Geometry check sheet. Reference: the model listing, model coordinates, mm. Face numbers are marked on the shaded views. Round coordinates to 2 decimals unless told otherwise and drop trailing zeros. Write each loop counter-clockwise with the first axis right and the second up, starting at its lowest first coordinate (ties: lowest second). Pieces come first, ordered by that corner, then holes.
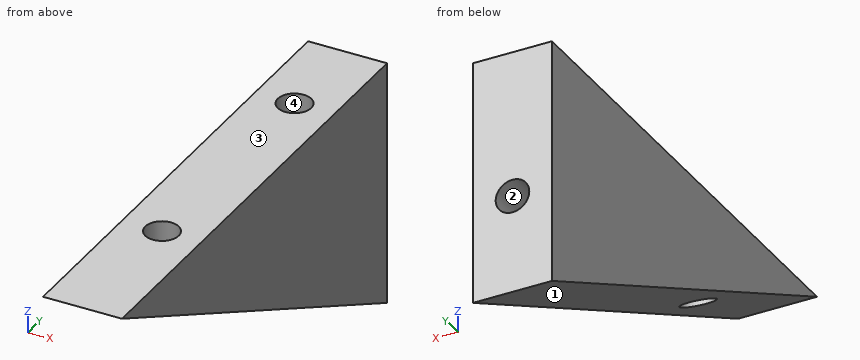
from build123d import *

# Parameters (mm, degrees)
EXTRUDE_1_DEPTH        = 16
HOLE_WIZARD_M8_1_D     = 6.8
HOLE_WIZARD_M8_1_DEPTH = 29.25
HOLE_WIZARD_M8_1_TIP   = 2.042926105
HOLE_WIZARD_M8_2_D     = 6.8
HOLE_WIZARD_M8_2_DEPTH = 29.25
HOLE_WIZARD_M8_2_TIP   = 2.042926105


with BuildPart() as part:
    # 草图1 → 凸台-拉伸1 (new body)
    with BuildSketch(Plane(origin=(0, 0, 0), x_dir=(0, 0, -1), z_dir=(1, 0, 0))):
        Polygon((0, 0), (50, 0), (0, -100), align=None)
    extrude(amount=EXTRUDE_1_DEPTH)

    # M8 螺纹孔1
    with Locations(Plane(origin=(0, 0, 0), x_dir=(1, 0, 0), z_dir=(0, 1, 0))):
        with Locations((8, 30)):
            Hole(HOLE_WIZARD_M8_1_D / 2, depth=HOLE_WIZARD_M8_1_DEPTH)
            with Locations((0, 0, -(HOLE_WIZARD_M8_1_DEPTH + HOLE_WIZARD_M8_1_TIP / 2))):  # 118° drill point
                Cone(0, HOLE_WIZARD_M8_1_D / 2, HOLE_WIZARD_M8_1_TIP, mode=Mode.SUBTRACT)

    # M8 螺纹孔2
    with Locations(Plane.XY):
        with Locations((8, -20), (8, -70)):
            Hole(HOLE_WIZARD_M8_2_D / 2, depth=HOLE_WIZARD_M8_2_DEPTH)
            with Locations((0, 0, -(HOLE_WIZARD_M8_2_DEPTH + HOLE_WIZARD_M8_2_TIP / 2))):  # 118° drill point
                Cone(0, HOLE_WIZARD_M8_2_D / 2, HOLE_WIZARD_M8_2_TIP, mode=Mode.SUBTRACT)


solid = part.part
1. Section check A-A (y = -13). Record the cut outline in (x, z).
2. Section check D-D (x = 1.5). Record the cut outline in (y, z).
3. Section check B-B (z = -23.5). Record the cut outline in (x, y), plus the area to 3 significant figures.
4. Release check for a two-part mould opening along Z. For the marked faces 1, 2, 3 and 4 record: +Z half, -Z half, draft (parallel to the pull), parting line (faces both ways), or undercut.
5. Section check C-C (y = -70). Record the cut outline in (x, z), plus the area to 3 significant figures.
6. Depth check by flat-ended pin: pin 1 Ø8 at (x, z) = (12, -21.5) entering from -Y; pin 2 Ø8 at (x, z) = (8, -30) entering from -Y; pin 3 Ø8 at (x, y) = (11, -30) entering from -Z; pin 4 Ø6 at (x, y) = (8, -70) entering from +Z. Enter the tip coordinate at first touch or a pass-through.
7. Scan lines: line 1 along Y through (x, z) = (8, -9.5); line 2 along X through (y, z) = (-7, -30); line 3 along Y through (x, z) = (8, -13). Record each from-to range of solid material in increasing order.
Results below:
1. outline: (0, -43.5) - (16, -43.5) - (16, 0) - (0, 0) - close; hole circle Ø6.8 at (8, -30)
2. outline: (-100, 0) - (0, -50) - (0, 0) - close
3. outline: (0, -53) - (16, -53) - (16, 0) - (0, 0) - close; hole circle Ø6.8 at (8, -20)
3. area: 812 mm2
4. face 1: -Z half
4. face 2: undercut
4. face 3: +Z half
4. face 4: draft
5. outline: (0, -15) - (4.6, -15) - (4.6, 0) - (0, 0) - close; (11.4, -15) - (16, -15) - (16, 0) - (11.4, 0) - close
5. area: 138 mm2
6. pin 1: stops at y = -65
6. pin 2: stops at y = -48
6. pin 3: stops at z = -37
6. pin 4: passes through
7. line 1: y = -81 to -73.4, -66.6 to -23.4, -16.6 to 0
7. line 2: x = 0 to 4.6, 11.4 to 16
7. line 3: y = -74 to -73.4, -66.6 to -23.4, -16.6 to 0
